```python
from build123d import *

# Parameters (mm, degrees)
MEMBER_40_X_3_1_DEPTH = 40


with BuildPart() as part:
    # Sketch1 → Member 40 X 3_1 (new body)
    with BuildSketch(Plane(origin=(0, 0, 0), x_dir=(0, 0, -1), z_dir=(1, 0, 0))):
        with BuildLine():
            Line((0, 0), (0, 40))
            Line((0, 40), (2, 40))
            ThreePointArc((2, 40), (2.707106781, 39.707106781), (3, 39))
            Line((3, 39), (3, 8))
            ThreePointArc((3, 8), (4.464466094, 4.464466094), (8, 3))
            Line((8, 3), (39, 3))
            ThreePointArc((39, 3), (39.707106781, 2.707106781), (40, 2))
            Line((40, 2), (40, 0))
            Line((40, 0), (0, 0))
        make_face()
    extrude(amount=MEMBER_40_X_3_1_DEPTH)


solid = part.part
```
The model under review builds one solid part; all positions refer to its coordinate system, in mm. A direction names the side the tool comes from. Coordinates: 2 decimals unless noted, no trailing zeros. Write each loop counter-clockwise with the first axis right and the second up, starting at its lowest first coordinate (ties: lowest second). Pieces come first, ordered by that corner, then holes.
1) We need section A-A on x = 37. State the section outline as (y, z) points.
2) We need section C-C on z = -28. State the section outline as (x, y) points.
3) Clearance check with flat-ended pins moving along their axes: pin 1 Ø1 at (x, y) = (27.5, 34.5) entering from +Z; pin 2 Ø2 at (x, y) = (32.5, 13) entering from -Z; pin 3 Ø8 at (x, z) = (16, -7.5) entering from +Y. State where each tip first meets the part, or that it passes through.
4) To check wall thickness, follow probe 1 along Y at (x, z) = (17, -17.5); probe 2 along Z at (x, y) = (22, 34.5); probe 3 along Y at (x, z) = (34.5, -5). State the ranges of each line that lie inside material, in increasing order.
5) We need section B-B on y = 21. State the section outline as (x, z) points.
6) Machinability: for faces 1 (the face through (20, 3, -23)), 2 (the face through (0, 2, -11)), which of the approach directions +Z, -Z, +X, -X, +Y, -Y give a long, thin tool a straight path to every point of the face, cutting with its end or side? Answer none if there is none.
Answer list:
1. outline: (0, -40) - (2, -40) arc R1 ccw to (3, -39) - (3, -8) arc R5 cw to (8, -3) - (39, -3) arc R1 ccw to (40, -2) - (40, 0) - (0, 0) - close
2. outline: (0, 0) - (40, 0) - (40, 3) - (0, 3) - close
3. pin 1: stops at z = 0
3. pin 2: stops at z = -3
3. pin 3: stops at y = 5.82
4. probe 1: y = 0 to 3
4. probe 2: z = -3 to 0
4. probe 3: y = 0 to 4
5. outline: (0, -3) - (40, -3) - (40, 0) - (0, 0) - close
6. face 1: -Z, +X, -X, +Y
6. face 2: +Z, -Z, -X, +Y, -Y
